Build history of the part. All positions in model axes, mm. Face numbers are marked on the shaded views. A direction names the side the tool comes from. Coordinates: 2 decimals unless noted, no trailing zeros. Order: outer loops, then holes, each group sorted by start corner. A loop starts at its lowest first (then second) coordinate and runs counter-clockwise, first axis right, second up. Notation, with made-up numbers: (-3.75, 75.5) - (10.25, 75.5) arc R24 ccw to (10.25, 99.5) - close; hole circle Ø6 at (-28, -15). An arc over 180 degrees is marked (long way). One line per item, written item: value.
from build123d import *

# Parameters (mm, degrees)
SKETCH_1_W            = 1140
SKETCH_1_H            = 1260
EXTRUDE_1_DEPTH       = 50
SKETCH_2_R            = 5
SKETCH_2_R_2          = 5.5
SKETCH_2_W            = 300
SKETCH_2_H            = 300
CUT_EXTRUDE_986_DEPTH = 20


with BuildPart() as part:
    # 草图1 → 凸台-拉伸1 (new body)
    with BuildSketch(Plane.XY):
        Rectangle(SKETCH_1_W, SKETCH_1_H)
    extrude(amount=EXTRUDE_1_DEPTH)

    # 草图2 → Cut-Extrude 986 (cut)
    with BuildSketch(Plane.XY.offset(50)):
        with Locations((0, -130)):
            Circle(SKETCH_2_R)
        with Locations((557.5, -530)):
            Circle(SKETCH_2_R_2)
        with Locations((557.5, 0)):
            Circle(SKETCH_2_R_2)
        with Locations((557.5, 530)):
            Circle(SKETCH_2_R_2)
        with Locations(Location((-557.5, 530, 0), (0, 0, 180))):
            Circle(SKETCH_2_R_2)
        with Locations(Location((-557.5, 0, 0), (0, 0, 180))):
            Circle(SKETCH_2_R_2)
        with Locations(Location((-557.5, -530, 0), (0, 0, 180))):
            Circle(SKETCH_2_R_2)
        with Locations((0, 630)):
            Rectangle(SKETCH_2_W, SKETCH_2_H)
    extrude(amount=-CUT_EXTRUDE_986_DEPTH, mode=Mode.SUBTRACT)


solid = part.part
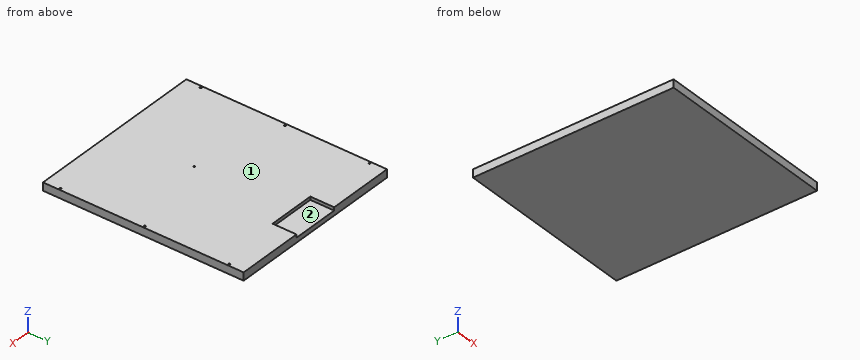
1. Band-saw the part on A-A, the plane z = 39. Give the cut face in (x, y).
Values found:
outline: (-570, -630) - (570, -630) - (570, 630) - (150, 630) - (150, 480) - (-150, 480) - (-150, 630) - (-570, 630) - close; hole circle Ø11 at (-557.5, -530); hole circle Ø11 at (-557.5, 0); hole circle Ø11 at (-557.5, 530); hole circle Ø10 at (0, -130); hole circle Ø11 at (557.5, -530); hole circle Ø11 at (557.5, 0); hole circle Ø11 at (557.5, 530)
2. Flat gauge pins, fed straight in: P1, Ø5.5, axis at x = 555, y = 531, coming from the +Z side; P2, Ø10, axis at x = 24.5, z = 38, coming from the +Y side. Where does each tip first touch, or does it go through?
Values found:
P1: stops at z = 30
P2: stops at y = 480
3. 3-axis set-ups, long thin cutter, end or side, ignore diameter. For the marked faces 1 and 2: which of +Z, -Z, +X, -X, +Y, -Y reach the whole face in a straight line?
Values found:
face 1: +Z, +X, -X, +Y, -Y
face 2: +Z, +Y
4. Band-saw the part on B-B, the plane x = -105.5. Give the cut face in (y, z), and give its area (3 significant figures).
Values found:
outline: (-630, 0) - (630, 0) - (630, 30) - (480, 30) - (480, 50) - (-630, 50) - close
area: 60,000 mm2
5. Probe line 1 along Y through (x, z) = (557.5, 41.5); line 2 along X through (y, z) = (-530, 43); line 3 along X through (y, z) = (530, 37.5). List the from-to ranges inside material, lowest first.
Values found:
line 1: y = -630 to -535.5, -524.5 to -5.5, 5.5 to 524.5, 535.5 to 630
line 2: x = -570 to -563, -552 to 552, 563 to 570
line 3: x = -570 to -563, -552 to -150, 150 to 552, 563 to 570
